The model under review builds one solid part; all positions refer to its coordinate system, in mm. Face numbers are marked on the shaded views. A direction names the side the tool comes from. Round coordinates to 2 decimals unless told otherwise and drop trailing zeros. Order: outer loops, then holes, each group sorted by start corner. A loop starts at its lowest first (then second) coordinate and runs counter-clockwise, first axis right, second up. Notation, with made-up numbers: M 77.5,-31 L 109.5,-31 A16 ccw 109.5,-15 Z; hole C 32.25,50 d3. An arc over 180 degrees is marked long. Answer as a JSON object with one key per item and string values. Group by question number.
1. Add section C-C on y = 16. State the section outline as (x, z) points.
2. Add section A-A on x = 0. Give the number of separate pieces and of enclosed holes in the cut face, and give its area (3 significant figures).
3. Clearance check with flat-ended pins moving along their axes: P1, Ø5, axis at x = -5, z = -1, coming from the +Y side; P2, Ø8, axis at x = 2, y = 13.5, coming from the +Z side; P3, Ø4, axis at x = -3.5, y = 22, coming from the +Z side. State where each tip first meets the part, or that it passes through.
4. Mouldability with a two-part tool opening along X and no side actions: class the marked faces 3, 4 and 5 as released by +X, released by -X, zero draft, split by the parting line, or undercut.
5. To check wall thickness, follow probe 1 along X at (y, z) = (2.5, 0); probe 2 along Y at (x, z) = (14, 3.5); probe 3 along Z at (x, y) = (-3, 10.25). State the ranges of each line that lie inside material, in increasing order. Write a range as [from, to].
6. Machinability: for the marked faces 1 and 2, which of the approach directions +Z, -Z, +X, -X, +Y, -Y give a long, thin tool a straight path to every point of the face, cutting with its end or side? Answer none if there is none.
```python
from build123d import *

# Parameters (mm, degrees)
SKETCH1_R           = 25
BOSS_EXTRUDE2_DEPTH = 5
SKETCH3_R           = 3
CUT_EXTRUDE2_DEPTH  = 5
SKETCH4_R           = 11
SKETCH4_R_2         = 8
BOSS_EXTRUDE3_DEPTH = 20
CHAMFER1_SIZE       = 0.8
FILLET1_R           = 1


with BuildPart() as part:
    # Sketch1 → Boss-Extrude2 (new body)
    with BuildSketch(Plane(origin=(0, 0, 0), x_dir=(1, 0, 0), z_dir=(0, 1, 0))):
        with Locations(Location((0, 0, 0), (0, 0, 270))):
            Circle(SKETCH1_R)
    extrude(amount=BOSS_EXTRUDE2_DEPTH)

    # Sketch3 → Cut-Extrude2 (cut)
    with BuildSketch(Plane(origin=(0, 0, 0), x_dir=(1, 0, 0), z_dir=(0, 1, 0))):
        with Locations(Location((-17.5, 0, 0), (0, 0, 270))):
            Circle(SKETCH3_R)
        with Locations(Location((0, 17.5, 0), (0, 0, 270))):
            Circle(SKETCH3_R)
        with Locations(Location((17.5, 0, 0), (0, 0, 270))):
            Circle(SKETCH3_R)
        with Locations(Location((0, -17.5, 0), (0, 0, 270))):
            Circle(SKETCH3_R)
    extrude(amount=CUT_EXTRUDE2_DEPTH, mode=Mode.SUBTRACT)

    # Sketch4 → Boss-Extrude3 (add)
    with BuildSketch(Plane(origin=(0, 5, 0), x_dir=(1, 0, 0), z_dir=(0, 1, 0))):
        with Locations(Location((0, 0, 0), (0, 0, 270))):
            Circle(SKETCH4_R)
        with Locations(Location((0, 0, 0), (0, 0, 270))):
            Circle(SKETCH4_R_2, mode=Mode.SUBTRACT)
    extrude(amount=BOSS_EXTRUDE3_DEPTH)

    # Chamfer1
    chamfer1_edges = [part.edges().sort_by_distance(p)[0] for p in [
        (0, 0, -25),
        (0, 25, -11),
        (0, 25, -8),
        (0, 5, -25),
    ]]
    chamfer(chamfer1_edges, length=CHAMFER1_SIZE)

    # Fillet1
    fillet1_edges = [part.edges().sort_by_distance(p)[0] for p in [
        (0, 5, -11),
    ]]
    fillet(fillet1_edges, radius=FILLET1_R)


solid = part.part
```
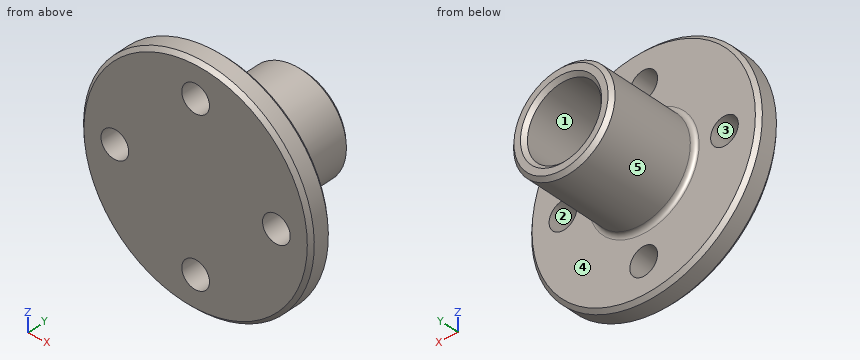
Recorded:
{
 "1": {"outline": "C 0,0 d22; hole C 0,0 d16"},
 "2": {"separate pieces": "3", "enclosed holes": "0", "area": "308 mm²"},
 "3": {"P1": "stops at y = 5", "P2": "stops at z = 11", "P3": "stops at z = 10.9"},
 "4": {"face 3": "undercut", "face 4": "zero draft", "face 5": "split by the parting line"},
 "5": {"probe 1": "x = [-25, -20.5], [-14.5, 14.5], [20.5, 25]", "probe 2": "y = [0, 5]", "probe 3": "z = [-10.58, -7.42], [7.42, 10.58]"},
 "6": {"face 1": "+Y", "face 2": "+Y, -Y"}
}
